Work out the finished part from the listing and answer in its coordinate system (mm). Face numbers are marked on the shaded views. A direction names the side the tool comes from. Coordinates: 2 decimals unless noted, no trailing zeros. Write each loop counter-clockwise with the first axis right and the second up, starting at its lowest first coordinate (ties: lowest second). Pieces come first, ordered by that corner, then holes. Notation, with made-up numbers: (22.25, 7) - (47.25, 7) arc R23 cw to (47.25, 36) - close; hole circle Ø10 at (20.5, -7). An arc over 180 degrees is marked (long way). Use a Markdown table: item, result. Add a question column.
(1) For a pull along X with two mould halves and no side action, classify the marked faces 3, 4, 5 and 6 as released by +X, released by -X, zero draft, split by the parting line, or undercut.
(2) The part is cut by section B-B, the plane y = -4. Give the vertices of the cut face in (x, z).
(3) A tool of negligible diameter and unlimited length cuts with its end or side. For the marked faces 1 and 2, from which of +Z, -Z, +X, -X, +Y, -Y can it reach the whole face along a straight path? Write none if from no direction.
(4) The part is cut by section D-D, the plane x = -12. Give the vertices of the cut face in (y, z), then the cut area to 3 significant figures.
(5) The part is cut by section C-C, the plane y = -24.5. Give the vertices of the cut face in (x, z).
(6) The part is cut by section A-A, the plane x = 0. Give the vertices of the cut face in (y, z).
(7) Find the intervals of material crossed by line 1 (Y direction, x = -12, z = -3); line 2 (Y direction, x = 8, z = 1.25); line 3 (Y direction, x = 12, z = 1.5), in increasing order. Write a range as from..to.
(8) Given pin 1 Ø5 at (x, z) = (-4.5, -3) entering from -Y; pin 2 Ø2.5 at (x, y) = (12, -24.5) entering from -Z, each flat-ended and moving along its own axis, determine where each tip first touches the part or whether it passes through.
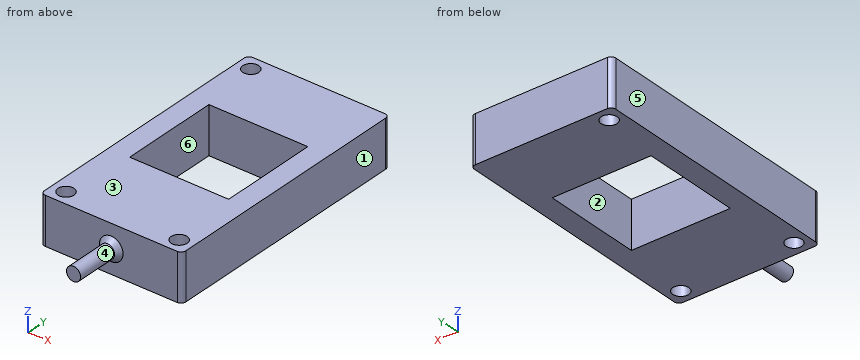
from build123d import *

# Parameters (mm, degrees)
SKETCH1_W                  = 30
SKETCH1_H                  = 55
BOSS_EXTRUDE1_DEPTH        = 5
SKETCH2_W                  = 21
SKETCH2_H                  = 21
CUT_EXTRUDE1_DEPTH         = 33.882366095
SKETCH3_R                  = 1.5
BOSS_EXTRUDE2_DEPTH        = 10
CHAMFER1_SIZE              = 1
FILLET1_R                  = 1
F_3_4_3_4_DIAMETER_HOLE1_D = 3.4


with BuildPart() as part:
    # Sketch1 → Boss-Extrude1 (new, symmetric)
    with BuildSketch(Plane.XY):
        Rectangle(SKETCH1_W, SKETCH1_H)
    extrude(amount=BOSS_EXTRUDE1_DEPTH, both=True)

    # Sketch2 → Cut-Extrude1 (cut, through all)
    with BuildSketch(Plane.XY.offset(5)):
        with Locations((0, 1)):
            Rectangle(SKETCH2_W, SKETCH2_H)
    extrude(amount=-CUT_EXTRUDE1_DEPTH, mode=Mode.SUBTRACT)

    # Sketch3 → Boss-Extrude2 (add)
    with BuildSketch(Plane.XZ.offset(27.5)):
        with Locations(Location((0, 0, 0), (0, 0, 90))):
            Circle(SKETCH3_R)
    extrude(amount=BOSS_EXTRUDE2_DEPTH)

    # Chamfer1
    chamfer1_edges = [part.edges().sort_by_distance(p)[0] for p in [
        (0, -27.5, -1.5),
    ]]
    chamfer(chamfer1_edges, length=CHAMFER1_SIZE)

    # Fillet1
    fillet1_edges = [part.edges().sort_by_distance(p)[0] for p in [
        (15, -27.5, 0),
        (-15, -27.5, 0),
        (-15, 27.5, 0),
        (15, 27.5, 0),
    ]]
    fillet(fillet1_edges, radius=FILLET1_R)

    # Ø3.4 (3.4) Diameter Hole1 (through all)
    with Locations(Plane.XY.offset(5)):
        with Locations((-12, 24.5), (-12, -24.5), (12, -24.5)):
            Hole(F_3_4_3_4_DIAMETER_HOLE1_D / 2)


solid = part.part
Model answer:
| question | item | result |
|---|---|---|
| 1 | face 3 | zero draft |
| 1 | face 4 | split by the parting line |
| 1 | face 5 | released by -X |
| 1 | face 6 | undercut |
| 2 | outline | (-15, -5) - (-10.5, -5) - (-10.5, 5) - (-15, 5) - close; (10.5, -5) - (15, -5) - (15, 5) - (10.5, 5) - close |
| 3 | face 1 | +Z, -Z, +X, +Y, -Y |
| 3 | face 2 | +Z, -Z |
| 4 | outline | (-27.5, -5) - (-26.2, -5) - (-26.2, 5) - (-27.5, 5) - close; (-22.8, -5) - (22.8, -5) - (22.8, 5) - (-22.8, 5) - close; (26.2, -5) - (27.5, -5) - (27.5, 5) - (26.2, 5) - close |
| 4 | area | 482 mm^2 |
| 5 | outline | (-15, -5) - (-13.7, -5) - (-13.7, 5) - (-15, 5) - close; (-10.3, -5) - (10.3, -5) - (10.3, 5) - (-10.3, 5) - close; (13.7, -5) - (15, -5) - (15, 5) - (13.7, 5) - close |
| 6 | outline | (-37.5, -1.5) - (-28.5, -1.5) - (-27.5, -2.5) - (-27.5, -5) - (-9.5, -5) - (-9.5, 5) - (-27.5, 5) - (-27.5, 2.5) - (-28.5, 1.5) - (-37.5, 1.5) - close; (11.5, -5) - (27.5, -5) - (27.5, 5) - (11.5, 5) - close |
| 7 | line 1 | -27.5..-26.2, -22.8..22.8, 26.2..27.5 |
| 7 | line 2 | -27.5..-9.5, 11.5..27.5 |
| 7 | line 3 | -27.5..-26.2, -22.8..27.5 |
| 8 | pin 1 | y = -27.5 |
| 8 | pin 2 | through |
